```python
from build123d import *

# Parameters (mm, degrees)
SKETCH_1_W                = 100
SKETCH_1_H                = 136
EXTRUDE_1_DEPTH           = 4
SKETCH_3_W                = 75
SKETCH_3_H                = 15
EXTRUDE_2_DEPTH           = 4
CHAMFER_2_SIZE            = 7.7
CHAMFER_2_SIZE2           = 1.4
CHAMFER_3_SIZE            = 1.4
CHAMFER_3_SIZE2           = 7.7
FILLET_1_R                = 5
CHAMFER_4_SIZE            = 3
HOLE_WIZARD_M4_1_D        = 3.3
HOLE_WIZARD_M4_1_DEPTH    = 11.5
HOLE_WIZARD_M4_1_TIP      = 0.991420021
SKETCH_8_W                = 362.353371429
SKETCH_8_H                = 115.701942857
CUT_EXTRUDE_4_DEPTH       = 114.877126764
CHAMFER_5_SIZE            = 3
HOLE_WIZARD_1_D           = 4.5
HOLE_WIZARD_1_CBORE_D     = 8
HOLE_WIZARD_1_CBORE_DEPTH = 5
CHAMFER_6_SIZE            = 3
SKETCH_14_W               = 127.06003401
SKETCH_14_H               = 84.591980831
CUT_EXTRUDE_5_DEPTH       = 43
SKETCH_15_R               = 2.5
CUT_EXTRUDE_6_DEPTH       = 16.5


with BuildPart() as part:
    # 草图1 → 凸台-拉伸1 (new, symmetric)
    with BuildSketch(Plane.XY):
        with Locations((0, -34)):
            Rectangle(SKETCH_1_W, SKETCH_1_H)
    extrude(amount=EXTRUDE_1_DEPTH, both=True)

    # 草图3 → 凸台-拉伸2 (add, symmetric)
    with BuildSketch(Plane.XY):
        with Locations((0, 41.5)):
            Rectangle(SKETCH_3_W, SKETCH_3_H)
    extrude(amount=EXTRUDE_2_DEPTH, both=True)

    # 倒角2
    chamfer_2_edges = [part.edges().sort_by_distance(p)[0] for p in [
        (-37.5, 49, 0),
    ]]
    chamfer_2_side = [part.faces().sort_by_distance(p)[0] for p in [
        (0, 49, 0),
    ]]
    chamfer(chamfer_2_edges, length=CHAMFER_2_SIZE, length2=CHAMFER_2_SIZE2, reference=chamfer_2_side[0])

    # 倒角3
    chamfer_3_edges = [part.edges().sort_by_distance(p)[0] for p in [
        (37.5, 49, 0),
    ]]
    chamfer_3_side = [part.faces().sort_by_distance(p)[0] for p in [
        (37.5, 41.5, 0),
    ]]
    chamfer(chamfer_3_edges, length=CHAMFER_3_SIZE, length2=CHAMFER_3_SIZE2, reference=chamfer_3_side[0])

    # 圆角1
    fillet_1_edges = [part.edges().sort_by_distance(p)[0] for p in [
        (-37.5, 34, 0),
        (37.5, 34, 0),
    ]]
    fillet(fillet_1_edges, radius=FILLET_1_R)

    # 倒角4
    chamfer_4_edges = [part.edges().sort_by_distance(p)[0] for p in [
        (50, -102, 0),
        (-50, -102, 0),
    ]]
    chamfer(chamfer_4_edges, length=CHAMFER_4_SIZE)

    # M4 螺纹孔1
    with Locations(Plane(origin=(0, 49, 0), x_dir=(1, 0, 0), z_dir=(0, 1, 0))):
        with Locations((-20, 0), (20, 0)):
            Hole(HOLE_WIZARD_M4_1_D / 2, depth=HOLE_WIZARD_M4_1_DEPTH)
            with Locations((0, 0, -(HOLE_WIZARD_M4_1_DEPTH + HOLE_WIZARD_M4_1_TIP / 2))):  # 118° drill point
                Cone(0, HOLE_WIZARD_M4_1_D / 2, HOLE_WIZARD_M4_1_TIP, mode=Mode.SUBTRACT)

    # 草图8 → 切除-拉伸4 (cut, through all)
    with BuildSketch(Plane(origin=(0, 0, -4), x_dir=(-1, 0, 0), z_dir=(0, 0, -1))):
        with Locations((78.704228572, -69.850971429)):
            Rectangle(SKETCH_8_W, SKETCH_8_H)
    extrude(amount=-CUT_EXTRUDE_4_DEPTH, mode=Mode.SUBTRACT)

    # 倒角5
    chamfer_5_edges = [part.edges().sort_by_distance(p)[0] for p in [
        (-50, -12, 0),
        (50, -12, 0),
    ]]
    chamfer(chamfer_5_edges, length=CHAMFER_5_SIZE)

    # 打孔尺寸(%根据)开槽圆柱头螺钉的类型1 (through all)
    with Locations(Plane.XY.offset(4)):
        with Locations((-43.15, -3), (43.15, -3), (-45, 29), (45, 29)):
            CounterBoreHole(HOLE_WIZARD_1_D / 2, HOLE_WIZARD_1_CBORE_D / 2, HOLE_WIZARD_1_CBORE_DEPTH)

    # 倒角6
    chamfer_6_edges = [part.edges().sort_by_distance(p)[0] for p in [
        (-50, 34, 0),
        (50, 34, 0),
    ]]
    chamfer(chamfer_6_edges, length=CHAMFER_6_SIZE)

    # 草图14 → 切除-拉伸5 (cut)
    with BuildSketch(Plane.XY.offset(4)):
        with Locations((-7.727502701, 2.704009584)):
            Rectangle(SKETCH_14_W, SKETCH_14_H)
    extrude(amount=-CUT_EXTRUDE_5_DEPTH, mode=Mode.SUBTRACT)

    # 草图15 → 切除-拉伸6 (cut)
    with BuildSketch(Plane(origin=(0, 49, 0), x_dir=(1, 0, 0), z_dir=(0, 1, 0))):
        with Locations(Location((-20, 0, 0), (0, 0, 270))):
            Circle(SKETCH_15_R)
        with Locations(Location((20, 0, 0), (0, 0, 270))):
            Circle(SKETCH_15_R)
    extrude(amount=-CUT_EXTRUDE_6_DEPTH, mode=Mode.SUBTRACT)


solid = part.part
```
Build history of the part. All positions in model axes, mm. Round coordinates to 2 decimals unless told otherwise and drop trailing zeros. Write each loop counter-clockwise with the first axis right and the second up, starting at its lowest first coordinate (ties: lowest second). Pieces come first, ordered by that corner, then holes. Notation, with made-up numbers: (49.5, 82) -> (97.5, 82) arc R29 cw to (97.5, 112) -> close; hole circle Ø11 at (71, -20.75). An arc over 180 degrees is marked (long way). Put each result on its own line as item: value.
Item 1: Slice it at C-C, the plane y = 45.6. Give the cut face in (x, z).
Here are the results:
outline: (-37.5, -4) -> (37.5, -4) -> (37.5, 4) -> (-37.5, 4) -> close; hole circle Ø5 at (-20, 0); hole circle Ø5 at (20, 0)
Item 2: Slice it at A-A, the plane x = 20. Give the cut face in (y, z).
Here are the results:
outline: (45, -4) -> (49, -4) -> (49, -2.5) -> (45, -2.5) -> close; (45, 2.5) -> (49, 2.5) -> (49, 4) -> (45, 4) -> close
Item 3: Two-plate mould, pull along Z, no slides. Class faces 1 (the face through (-1, 45, 0)), 2 (the face through (-17.52, 47.03, -0.33)), 3 (the face through (-1, 47, -4)), 4 (the face through (-1, 47, 4)): pulls with the +Z half, pulls with the -Z half, needs draft (parallel to the pull), parting line crosses it, or undercut.
Here are the results:
face 1: needs draft
face 2: undercut
face 3: pulls with the -Z half
face 4: pulls with the +Z half
Item 4: Slice it at D-D, the plane x = -30.5. Give the cut face in (y, z).
Here are the results:
outline: (45, -4) -> (48.87, -4) -> (48.87, 4) -> (45, 4) -> close
Item 5: Slice it at B-B, the plane z = 0. Give the cut face in (x, y).
Here are the results:
outline: (-37.5, 45) -> (-22.5, 45) -> (-22.5, 49) -> (-29.8, 49) -> (-37.5, 47.6) -> close; (-17.5, 45) -> (17.5, 45) -> (17.5, 49) -> (-17.5, 49) -> close; (22.5, 45) -> (37.5, 45) -> (37.5, 47.6) -> (29.8, 49) -> (22.5, 49) -> close
Item 6: Wall check: probe 1 along X at (y, z) = (46.7, 0); probe 2 along X at (y, z) = (46.7, -1.75); probe 3 along Z at (x, y) = (-18.5, 45.55). Give the ranges that are in metal, low to high. Write a range as from..to.
Here are the results:
probe 1: x = -37.5..-22.5, -17.5..17.5, 22.5..37.5
probe 2: x = -37.5..-21.79, -18.21..18.21, 21.79..37.5
probe 3: z = -4..-2, 2..4
